Drawing for the job (mm, zero at the part's lowest x, y, z). Round coordinates to 2 decimals unless told otherwise and drop trailing zeros. Write each loop counter-clockwise with the first axis right and the second up, starting at its lowest first coordinate (ties: lowest second). Pieces come first, ordered by that corner, then holes. Notation, with made-up numbers: M 72.25,0 L 126.25,0 A35 ccw 126.25,32 Z; hole C -4,-14 d4. An arc over 180 degrees is marked long. Use a Markdown table: item, result. Add a question column.
1) Slice it at C-C on x = 20. Write the cut outline in (y, z), plus the area to 3 significant figures.
2) Drop a flat-ended pin along its axis: P1, Ø10, axis at x = 20, y = 195, coming from the +Z side. Give the stop position or say it passes through.
3) Wall check: probe 1 along Y at (x, z) = (20, 7); probe 2 along Y at (x, z) = (15.5, 15.25); probe 3 along X at (y, z) = (195.5, 10). Give the ranges that are in metal, low to high.
4) Slice it at B-B on y = 270. Write the cut outline in (x, z), plus the area to 3 significant figures.
5) Slice it at A-A on z = 14.75. Write the cut outline in (x, y), plus the area to 3 significant figures.
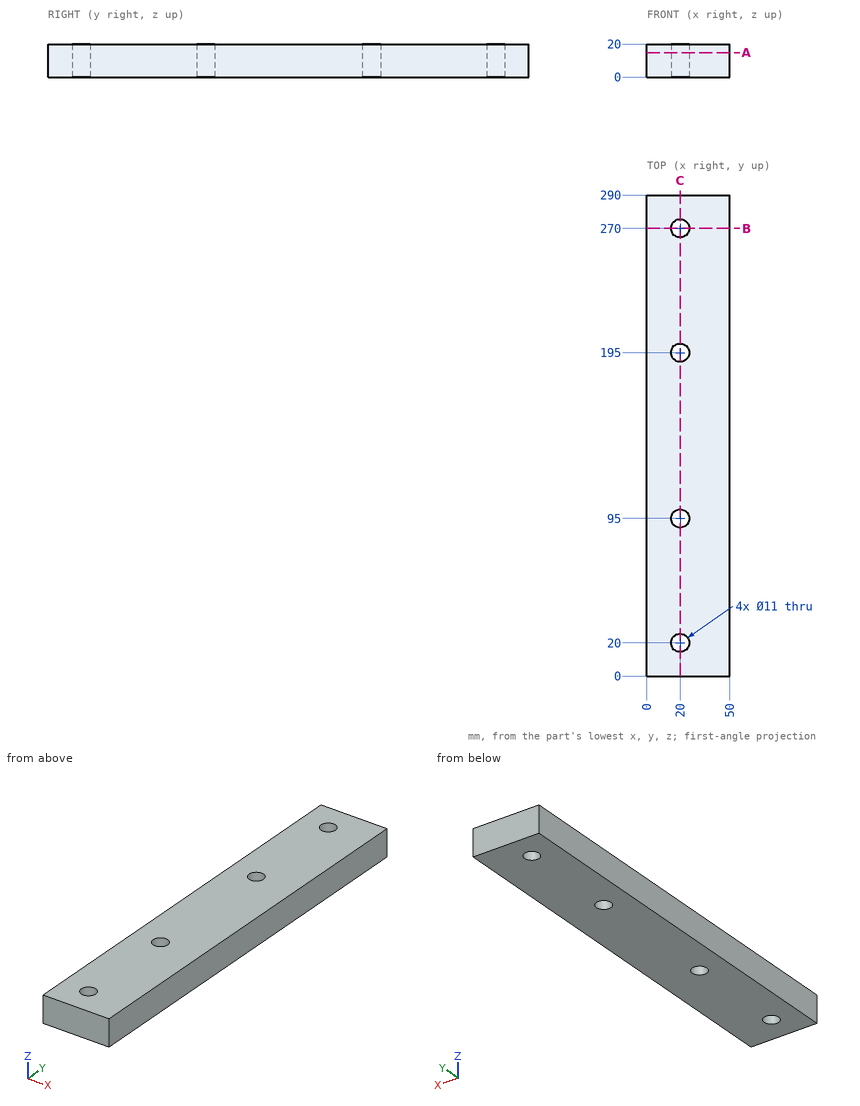
Entries:
| question | item | result |
|---|---|---|
| 1 | outline | M 0,0 L 14.5,0 L 14.5,20 L 0,20 Z; M 25.5,0 L 89.5,0 L 89.5,20 L 25.5,20 Z; M 100.5,0 L 189.5,0 L 189.5,20 L 100.5,20 Z; M 200.5,0 L 264.5,0 L 264.5,20 L 200.5,20 Z; M 275.5,0 L 290,0 L 290,20 L 275.5,20 Z |
| 1 | area | 4,920 mm^2 |
| 2 | P1 | passes through |
| 3 | probe 1 | y = 0 to 14.5, 25.5 to 89.5, 100.5 to 189.5, 200.5 to 264.5, 275.5 to 290 |
| 3 | probe 2 | y = 0 to 16.84, 23.16 to 91.84, 98.16 to 191.84, 198.16 to 266.84, 273.16 to 290 |
| 3 | probe 3 | x = 0 to 14.52, 25.48 to 50 |
| 4 | outline | M 0,0 L 14.5,0 L 14.5,20 L 0,20 Z; M 25.5,0 L 50,0 L 50,20 L 25.5,20 Z |
| 4 | area | 780 mm^2 |
| 5 | outline | M 0,0 L 50,0 L 50,290 L 0,290 Z; hole C 20,20 d11; hole C 20,95 d11; hole C 20,195 d11; hole C 20,270 d11 |
| 5 | area | 14,100 mm^2 |
